Model file for the job. Use its own axes, mm. Face numbers are marked on the shaded views. A direction names the side the tool comes from. Coordinates: 2 decimals unless noted, no trailing zeros. Order: outer loops, then holes, each group sorted by start corner. A loop starts at its lowest first (then second) coordinate and runs counter-clockwise, first axis right, second up.
from build123d import *

# Parameters (mm, degrees)
SKETCH1_W                = 120
SKETCH1_H                = 60
BOSS_EXTRUDE1_DEPTH      = 12
M6_CLEARANCE_HOLE1_D     = 9
M6_CLEARANCE_HOLE1_DEPTH = 32.75
M6_CLEARANCE_HOLE1_TIP   = 2.703872786
SKETCH3_W                = 120
SKETCH3_H                = 20
BOSS_EXTRUDE2_DEPTH      = 40
FILLET1_R                = 5


with BuildPart() as part:
    # Sketch1 → Boss-Extrude1 (new body)
    with BuildSketch(Plane.XY):
        with Locations((60, 30)):
            Rectangle(SKETCH1_W, SKETCH1_H)
    extrude(amount=BOSS_EXTRUDE1_DEPTH)

    # M6 Clearance Hole1
    with Locations(Plane(origin=(0, 0, 0), x_dir=(-1, 0, 0), z_dir=(0, 0, -1))):
        with Locations((-110, 50), (-10, 50), (-10, 10), (-110, 10)):
            Hole(M6_CLEARANCE_HOLE1_D / 2, depth=M6_CLEARANCE_HOLE1_DEPTH)
            with Locations((0, 0, -(M6_CLEARANCE_HOLE1_DEPTH + M6_CLEARANCE_HOLE1_TIP / 2))):  # 118° drill point
                Cone(0, M6_CLEARANCE_HOLE1_D / 2, M6_CLEARANCE_HOLE1_TIP, mode=Mode.SUBTRACT)

    # Sketch3 → Boss-Extrude2 (add)
    with BuildSketch(Plane.XY):
        with Locations((60, 30)):
            Rectangle(SKETCH3_W, SKETCH3_H)
    extrude(amount=-BOSS_EXTRUDE2_DEPTH)

    # Fillet1
    fillet1_edges = [part.edges().sort_by_distance(p)[0] for p in [
        (60, 20, -40),
        (60, 40, -40),
    ]]
    fillet(fillet1_edges, radius=FILLET1_R)


solid = part.part
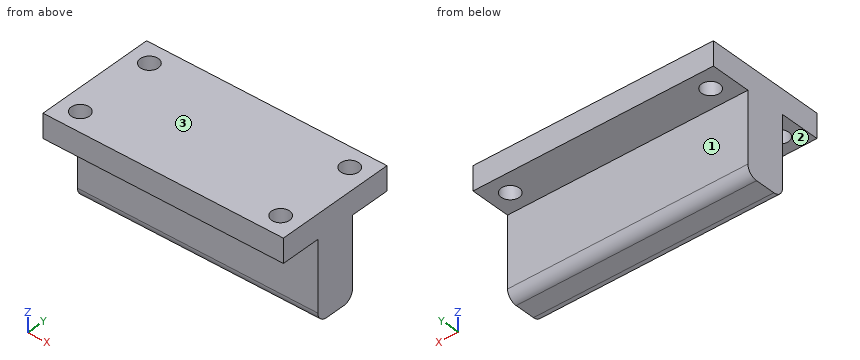
Q1. Cut at A-A, the plane x = 10. List the corners of the cut face in (y, z), plus the area to 3 significant figures.
Established:
outline: (0, 0) - (5.5, 0) - (5.5, 12) - (0, 12) - close; (14.5, 0) - (20, 0) - (20, -35) arc R5 ccw to (25, -40) - (35, -40) arc R5 ccw to (40, -35) - (40, 0) - (45.5, 0) - (45.5, 12) - (14.5, 12) - close; (54.5, 0) - (60, 0) - (60, 12) - (54.5, 12) - close
area: 1,290 mm2
Q2. Cut at C-C, the plane z = 6. List the corners of the cut face in (x, y).
Established:
outline: (0, 0) - (120, 0) - (120, 60) - (0, 60) - close; hole circle Ø9 at (10, 10); hole circle Ø9 at (10, 50); hole circle Ø9 at (110, 10); hole circle Ø9 at (110, 50)
Q3. Probe line 1 (Y direction, x = 10, z = 7.5); line 2 (X direction, y = 47.5, z = 8); line 3 (Z direction, x = 106, y = 56). List the from-to ranges inside material, lowest first.
Established:
line 1: y = 0 to 5.5, 14.5 to 45.5, 54.5 to 60
line 2: x = 0 to 6.26, 13.74 to 106.26, 113.74 to 120
line 3: z = 0 to 12
Q4. Cut at B-B, the plane y = 50. List the corners of the cut face in (x, z), plus the area to 3 significant figures.
Established:
outline: (0, 0) - (5.5, 0) - (5.5, 12) - (0, 12) - close; (14.5, 0) - (105.5, 0) - (105.5, 12) - (14.5, 12) - close; (114.5, 0) - (120, 0) - (120, 12) - (114.5, 12) - close
area: 1,220 mm2
Q5. Cut at D-D, the plane x = 48.5. List the corners of the cut face in (y, z), plus the area to 3 significant figures.
Established:
outline: (0, 0) - (20, 0) - (20, -35) arc R5 ccw to (25, -40) - (35, -40) arc R5 ccw to (40, -35) - (40, 0) - (60, 0) - (60, 12) - (0, 12) - close
area: 1,510 mm2
Q6. Which spindle directions (+Z, -Z, +X, -X, +Y, -Y) get a long thin tool onto all of the face, cutting with end or side? Do the marked faces 1, 2 and 3. Say none if no direction does.
Established:
face 1: -Z, +X, -X, +Y
face 2: -Z, +X, -X, -Y
face 3: +Z, +X, -X, +Y, -Y
Q7. Drop flat-ended pins along their axis: P1, Ø22, axis at x = 56, y = 13, coming from the -Z side; P2, Ø10.5, axis at x = 10, y = 10, coming from the -Z side; P3, Ø3, axis at x = 61, z = -33, coming from the -Y side. Give the stop position or say it passes through.
Established:
P1: stops at z = -39.9
P2: stops at z = 0
P3: stops at y = 20
